```python
from build123d import *

# Parameters (mm, degrees)
BASE_PLATE_DEPTH            = 10
UPRIGHT_WALL_DEPTH          = 50
CLEVIS_PIN_HOLE_SKETCH_R    = 6
CLEVIS_PIN_HOLE_DEPTH       = 50
CLEVIS_SLOT_SKETCH_W        = 24
CLEVIS_SLOT_SKETCH_H        = 20
CLEVIS_SLOT_DEPTH           = 25
PLATE_BORE_SKETCH_R         = 10
PLATE_BORE_DEPTH            = 10
GUSSET_RIB_DEPTH            = 50
RIB_TRIM_CUT_1_DEPTH        = 21
RIB_TRIM_CUT_2_DEPTH        = 21
SLOT_RELIEF_POCKET_SKETCH_W = 24
SLOT_RELIEF_POCKET_SKETCH_H = 20
SLOT_RELIEF_POCKET_DEPTH    = 5


with BuildPart() as part:
    # Base Plate Profile → Base Plate (new body)
    with BuildSketch(Plane.XY):
        Polygon((90, 0), (5, 0), (0, 5), (0, 45), (5, 50), (90, 50), align=None)
    extrude(amount=BASE_PLATE_DEPTH)

    # Upright Wall Profile → Upright Wall (add)
    with BuildSketch(Plane.XZ):
        Polygon((90, 10), (90, 50), (85, 55), (71, 55), (66, 50), (66, 10), align=None)
    extrude(amount=-UPRIGHT_WALL_DEPTH)

    # Clevis Pin Hole Sketch → Clevis Pin Hole (cut)
    with BuildSketch(Plane.XZ):
        with Locations(Location((78, 45, 0), (0, 0, 270))):
            Circle(CLEVIS_PIN_HOLE_SKETCH_R)
    extrude(amount=-CLEVIS_PIN_HOLE_DEPTH, mode=Mode.SUBTRACT)

    # Clevis Slot Sketch → Clevis Slot (cut)
    with BuildSketch(Plane.XY.offset(55)):
        with Locations((78, 25)):
            Rectangle(CLEVIS_SLOT_SKETCH_W, CLEVIS_SLOT_SKETCH_H)
    extrude(amount=-CLEVIS_SLOT_DEPTH, mode=Mode.SUBTRACT)

    # Plate Bore Sketch → Plate Bore (cut)
    with BuildSketch(Plane.XY.offset(10)):
        with Locations((21, 25)):
            Circle(PLATE_BORE_SKETCH_R)
    extrude(amount=-PLATE_BORE_DEPTH, mode=Mode.SUBTRACT)

    # Gusset Rib Profile → Gusset Rib (add)
    with BuildSketch(Plane.XZ):
        Polygon((66, 10), (66, 25), (31, 10), align=None)
    extrude(amount=-GUSSET_RIB_DEPTH)

    # Rib Trim Cut 1 Sketch → Rib Trim Cut 1 (cut)
    with BuildSketch(Plane.XZ):
        Polygon((66, 25), (66, 10), (31, 10), align=None)
    extrude(amount=-RIB_TRIM_CUT_1_DEPTH, mode=Mode.SUBTRACT)

    # Rib Trim Cut 2 Sketch → Rib Trim Cut 2 (cut)
    with BuildSketch(Plane(origin=(0, 50, 0), x_dir=(1, 0, 0), z_dir=(0, 1, 0))):
        Polygon((66, -25), (66, -10), (31, -10), align=None)
    extrude(amount=-RIB_TRIM_CUT_2_DEPTH, mode=Mode.SUBTRACT)

    # Slot Relief Pocket Sketch → Slot Relief Pocket (cut)
    with BuildSketch(Plane.XY.offset(30)):
        with Locations((78, 25)):
            Rectangle(SLOT_RELIEF_POCKET_SKETCH_W, SLOT_RELIEF_POCKET_SKETCH_H)
    extrude(amount=-SLOT_RELIEF_POCKET_DEPTH, mode=Mode.SUBTRACT)


solid = part.part
```
Source: CAD feature listing. Evaluate the final solid. Frame: model axes, mm. A direction names the side the tool comes from. Coordinates: 2 decimals unless noted, no trailing zeros. Loops run counter-clockwise (first coordinate to the right, second up) from the corner with the lowest first, then second, coordinate; pieces in that order, holes last. Notation, with made-up numbers: (-22.5, 32) - (0.5, 32) arc R11 cw to (0.5, 50) - close; hole circle Ø3 at (13, 32.25). An arc over 180 degrees is marked (long way). Answer as CSV lines item,"result".
1. Ray query, line 1 (X direction, y = 42.5, z = 45); line 2 (Y direction, x = 21, z = 6); line 3 (Z direction, x = 51, y = 18.5). Return the intervals inside material, ascending.
Established:
line 1,"x = 66 to 72, 84 to 90"
line 2,"y = 0 to 15, 35 to 50"
line 3,"z = 0 to 10"
2. Section D-D (z = 30.5). Return loops of the section in (x, y), then the cut area to 3 significant figures.
Established:
outline,"(66, 0) - (90, 0) - (90, 15) - (66, 15) - close; (66, 35) - (90, 35) - (90, 50) - (66, 50) - close"
area,"720 mm2"
3. Section A-A (x = 21). Return loops of the section in (y, z).
Established:
outline,"(0, 0) - (15, 0) - (15, 10) - (0, 10) - close; (35, 0) - (50, 0) - (50, 10) - (35, 10) - close"
4. Section B-B (z = 45). Return loops of the section in (x, y), then the cut area to 3 significant figures.
Established:
outline,"(66, 0) - (72, 0) - (72, 15) - (66, 15) - close; (66, 35) - (72, 35) - (72, 50) - (66, 50) - close; (84, 0) - (90, 0) - (90, 15) - (84, 15) - close; (84, 35) - (90, 35) - (90, 50) - (84, 50) - close"
area,"360 mm2"
5. Section C-C (y = 13). Return loops of the section in (x, z), then the cut area to 3 significant figures.
Established:
outline,"(0, 0) - (90, 0) - (90, 50) - (85, 55) - (71, 55) - (66, 50) - (66, 10) - (0, 10) - close; hole circle Ø12 at (78, 45)"
area,"1,840 mm2"
6. Mould query, pull axis Y, two halves, no side actions, for faces 1 (the flat face through (78, 35, 37)), 2 (the cylindrical face through (82.06, 7.4, 49.42)), 3 (the flat face through (56, 29, 14)). Classes: released by +Y, released by -Y, zero draft, split by the parting line, or undercut.
Established:
face 1,"undercut"
face 2,"zero draft"
face 3,"released by +Y"
7. Contact query for flat-ended pins moving along their axis: pin 1 (3 mm diameter, centred on x = 51.5, z = 19.5, fed in from +Y); pin 2 (18 mm diameter, centred on x = 21, y = 25, fed in from -Z); pin 3 (2 mm diameter, centred on x = 68.5, y = 45, fed in from +Z); pin 4 (4.5 mm diameter, centred on x = 44, z = 15, fed in from -Y). Output: stop coordinate, or through.
Established:
pin 1,"stops at y = 29"
pin 2,"passes through"
pin 3,"stops at z = 53.5"
pin 4,"stops at y = 21"
8. Reachability of faces 4 (the flat face through (66, 8, 30)), 5 (the flat face through (33, 31, 10)), 6 (the flat face through (69, 42, 53)), 7 (the flat face through (66, 42, 30)), 8 (the flat face through (78, 25, 25)) from +Z, -Z, +X, -X, +Y, -Y: full face, straight path, thin tool, end or side. Return the list, or none.
Established:
face 4,"+Z, -X, -Y"
face 5,"+Z, -X"
face 6,"+Z, -X, +Y, -Y"
face 7,"+Z, -X, +Y"
face 8,"+Z, +X, -X"
